The model under review builds one solid part; all positions refer to its coordinate system, in mm. Face numbers are marked on the shaded views. Give positions to 0.01 mm unless a question says otherwise; leave off trailing zeros. Order: outer loops, then holes, each group sorted by start corner. A loop starts at its lowest first (then second) coordinate and runs counter-clockwise, first axis right, second up. Notation, with made-up numbers: (86, 19.25) - (103, 19.25) arc R9 cw to (103, 35.25) - close; hole circle Ø7 at (4.5, 17). An arc over 180 degrees is marked (long way). Use CSV: the item, a comma, the result in double quotes.
```python
from build123d import *

# Parameters (mm, degrees)
SKETCH1_R           = 5.5
SKETCH1_R_2         = 6.36045924
SKETCH1_R_3         = 5.351214453
SKETCH1_R_4         = 5.079203988
BOSS_EXTRUDE1_DEPTH = 18
SKETCH2_R           = 35.389686151
BOSS_EXTRUDE2_DEPTH = 110


with BuildPart() as part:
    # Sketch1 → Boss-Extrude1 (new body)
    with BuildSketch(Plane(origin=(0, 0, 0), x_dir=(1, 0, 0), z_dir=(0, 1, 0))):
        Polygon((204.197706314, -490.073376619), (-225.802293686, -490.073376619), (-225.802293686, -290.073376619), (-225.802293686, 530.17461365), (204.197706314, 530.17461365), align=None)
        with Locations(Location((186.197706314, -475.073376619, 0), (0, 0, 270))):
            Circle(SKETCH1_R, mode=Mode.SUBTRACT)
        with Locations(Location((186.197706314, -305.073376619, 0), (0, 0, 270))):
            Circle(SKETCH1_R_2, mode=Mode.SUBTRACT)
        with Locations(Location((-207.802293686, -305.073376619, 0), (0, 0, 270))):
            Circle(SKETCH1_R_3, mode=Mode.SUBTRACT)
        with Locations(Location((-207.802293686, -475.073376619, 0), (0, 0, 270))):
            Circle(SKETCH1_R_4, mode=Mode.SUBTRACT)
    extrude(amount=BOSS_EXTRUDE1_DEPTH)

    # Sketch2 → Boss-Extrude2 (add)
    with BuildSketch(Plane.XZ):
        with Locations(Location((96.665522834, 393.073168436, 0), (0, 0, 90))):
            Circle(SKETCH2_R)
        with Locations(Location((-118.270110206, 393.073168436, 0), (0, 0, 90))):
            Circle(SKETCH2_R)
        with Locations(Location((-118.270110206, -433.174405466, 0), (0, 0, 90))):
            Circle(SKETCH2_R)
        with Locations(Location((96.665522834, -433.174405466, 0), (0, 0, 90))):
            Circle(SKETCH2_R)
    extrude(amount=BOSS_EXTRUDE2_DEPTH)


solid = part.part
```
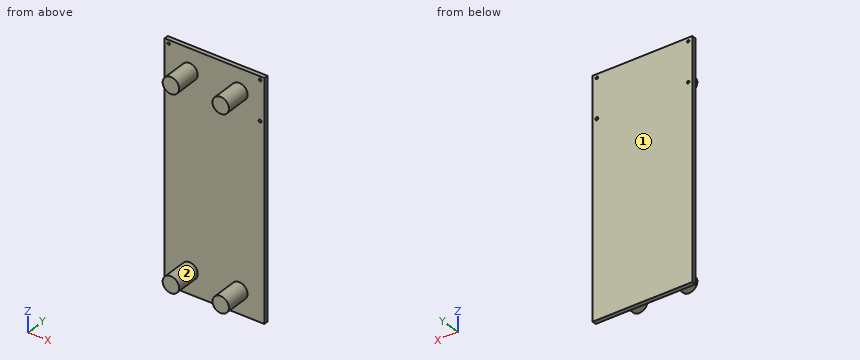
Item 1: Take a section at C-C, the plane x = -47. Give the boundary of the cut face in (y, z), and give its area (3 significant figures).
Results list:
outline,"(0, -530.17) - (18, -530.17) - (18, 490.07) - (0, 490.07) - close"
area,"18,400 mm2"
Item 2: Take a section at B-B, the plane z = -120.5. Give the boundary of the cut face in (x, y).
Results list:
outline,"(-225.8, 0) - (204.2, 0) - (204.2, 18) - (-225.8, 18) - close"
Item 3: Take a section at A-A, the plane y = -100.5. Give the boundary of the cut face in (x, z), and give its area (3 significant figures).
Results list:
outline,"circle Ø70.78 at (-118.27, -433.17); circle Ø70.78 at (-118.27, 393.07); circle Ø70.78 at (96.67, -433.17); circle Ø70.78 at (96.67, 393.07)"
area,"15,700 mm2"
Item 4: Wall thickness on L1, parallel to Y at x = -174, z = 412.5; L2, parallel to Z at x = -136, y = -103; L3, parallel to X at y = -59, z = 417: over which ranges is each line inside the solid? List them lowest first.
Results list:
L1,"y = 0 to 18"
L2,"z = -463.8 to -402.55, 362.45 to 423.7"
L3,"x = -144.35 to -92.19, 70.59 to 122.74"
Item 5: Mouldability with a two-part tool opening along Z and no side actions: class the marked faces 1 and 2 as pulls with the +Z half, pulls with the -Z half, needs draft (parallel to the pull), parting line crosses it, or undercut.
Results list:
face 1,"needs draft"
face 2,"undercut"
Item 6: Clearance check with flat-ended pins moving along their axes: pin 1 (20.5 mm diameter, centred on x = 186.2, z = 305.07, fed in from +Y); pin 2 (12.5 mm diameter, centred on x = -207.8, z = 305.07, fed in from -Y); pin 3 (3 mm diameter, centred on x = -122, y = -23.5, fed in from -Z); pin 4 (2 mm diameter, centred on x = -134.5, y = -43.5, fed in from -Z). State where each tip first meets the part, or that it passes through.
Results list:
pin 1,"stops at y = 18"
pin 2,"stops at y = 0"
pin 3,"stops at z = -468.49"
pin 4,"stops at z = -465.12"
